Geometry: final body of the model. Coordinates: model frame, mm. Face numbers are marked on the shaded views. A direction names the side the tool comes from. Give positions to 0.01 mm unless a question says otherwise; leave off trailing zeros. Loops run counter-clockwise (first coordinate to the right, second up) from the corner with the lowest first, then second, coordinate; pieces in that order, holes last. Notation, with made-up numbers: (17.5, 0.5) -> (26.5, 0.5) arc R26 ccw to (26.5, 36.5) -> close; hole circle Ø2 at (34, 54). An arc over 180 degrees is marked (long way). One line per question, with ' | ' between items. Start each with the question number.
Item 1: Section D-D on z = 71.5. Return loops of the section in (x, y), then the cut area to 3 significant figures.
Item 2: Mould query, pull axis X, two halves, no side actions, for the marked faces 3, 4, 5 and 6. Classes: released by +X, released by -X, zero draft, split by the parting line, or undercut.
Item 3: Pin query (flat end, axial travel): P1, Ø3, axis at y = 7, z = 33, coming from the +X side; P2, Ø3, axis at x = -2.5, z = 8, coming from the +Y side; P3, Ø6, axis at x = -5.5, z = 41, coming from the -Y side; P4, Ø5, axis at x = 0, y = 0, coming from the +Z side. Return the tip coordinate at first contact, or that it passes through.
Item 4: Section C-C on z = 39.5. Return loops of the section in (x, y).
Item 5: Material intervals for line 1 along Y through (x, z) = (0, 45); line 2 along Z through (x, y) = (2.5, -7.25); line 3 along Y through (x, z) = (0, 70.75), sorted ascending. Write a range as [from, to].
Item 6: Section B-B on z = 6. Return loops of the section in (x, y).
Item 7: Set-up query: the marked faces 1 and 2. Return all of +Z, -Z, +X, -X, +Y, -Y with unobstructed straight access to the full face (end or side cutting, diameter ignored); none if empty.
from build123d import *

# Parameters (mm, degrees)
SKETCH_1_R                 = 10
EXTRUDE_1_DEPTH            = 70
SKETCH_2_R                 = 5
EXTRUDE_2_DEPTH            = 10.5
SKETCH_3_W                 = 0.75
SKETCH_3_H                 = 2.5
SKETCH_4_R                 = 1.5
CUT_EXTRUDE_1_DEPTH        = 15.5
HOLE_WIZARD_6_0_6_1_REACH  = 68.521
HOLE_WIZARD_6_0_6_1_BORE_R = 3
CHAMFER_1_SIZE             = 0.5
SKETCH_9_W                 = 10
SKETCH_9_H                 = 12
CUT_EXTRUDE_2_DEPTH        = 1.5


with BuildPart() as part:
    # 草图1 → 凸台-拉伸1 (new body)
    with BuildSketch(Plane.XY):
        Circle(SKETCH_1_R)
    extrude(amount=EXTRUDE_1_DEPTH)

    # 草图2 → 凸台-拉伸2 (add)
    with BuildSketch(Plane.XY.offset(70)):
        with Locations(Location((0, 0, 0), (0, 0, 180))):
            Circle(SKETCH_2_R)
    extrude(amount=EXTRUDE_2_DEPTH)

    # 草图3 → 切除-旋转1 (revolve, cut)
    with BuildSketch(Plane(origin=(0, 0, 0), x_dir=(1, 0, 0), z_dir=(0, 1, 0)), mode=Mode.PRIVATE) as cut_revolve_1_sk:
        with Locations((-4.625, -71.25)):
            Rectangle(SKETCH_3_W, SKETCH_3_H)
    revolve(cut_revolve_1_sk.sketch.rotate(Axis((0, 0, 80.5), (0, 0, -1)), 180), axis=Axis((0, 0, 80.5), (0, 0, -1)), mode=Mode.SUBTRACT)

    # 草图4 → 切除-拉伸1 (cut)
    with BuildSketch(Plane.XY.offset(80.5)):
        Circle(SKETCH_4_R)
    extrude(amount=-CUT_EXTRUDE_1_DEPTH, mode=Mode.SUBTRACT)

    # 草图5 → 1/4 NPT 螺纹孔1 (revolve, cut)
    with BuildSketch(Plane.YZ):
        Polygon((0, 0), (0, 20.412347279), (5.5626, 17.07), (5.5626, 10.02), (5.943676082, 10.02), (6.2436883, 0), align=None)
    revolve(axis=Axis((0, 0, -6.35), (0, 0, 1)), mode=Mode.SUBTRACT)

    # Ø6.0 (6) 直径孔1 bore → Ø6.0 (6) 直径孔1 (cut, up to next)
    with BuildSketch(Plane.XY.offset(65), mode=Mode.PRIVATE) as hole_wizard_6_0_6_1_sk1:
        Circle(HOLE_WIZARD_6_0_6_1_BORE_R)
    hole_wizard_6_0_6_1_tool1 = extrude(hole_wizard_6_0_6_1_sk1.sketch, amount=-HOLE_WIZARD_6_0_6_1_REACH, mode=Mode.PRIVATE) & part.part
    add(hole_wizard_6_0_6_1_tool1.solids().sort_by_distance((0, 0, 65))[0], mode=Mode.SUBTRACT)

    # 倒角1
    chamfer_1_edges = [part.edges().sort_by_distance(p)[0] for p in [
        (-10, 0, 0),
        (-10, 0, 70),
        (5, 0, 80.5),
    ]]
    chamfer(chamfer_1_edges, length=CHAMFER_1_SIZE)

    # 草图9 → 切除-拉伸2 (cut)
    with BuildSketch(Plane(origin=(0, 10, 0), x_dir=(1, 0, 0), z_dir=(0, 1, 0))):
        with Locations((0, -6)):
            Rectangle(SKETCH_9_W, SKETCH_9_H)
    cut_extrude_2 = extrude(amount=-CUT_EXTRUDE_2_DEPTH, mode=Mode.SUBTRACT)

    # 镜向1: 切除-拉伸2 across plane
    add(cut_extrude_2.mirror(Plane.ZX), mode=Mode.SUBTRACT)


solid = part.part
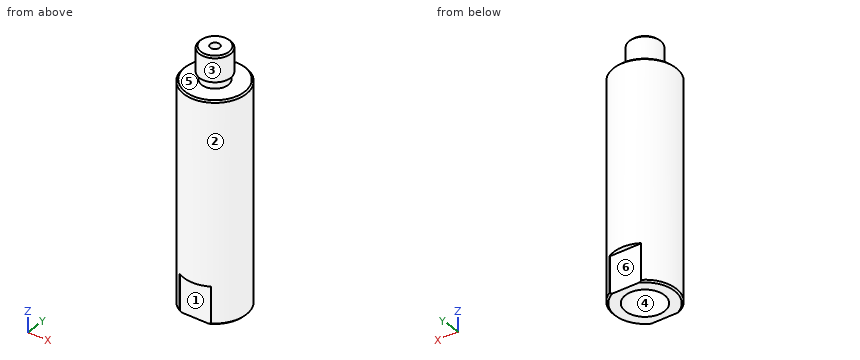
Result sheet:
1) outline: circle Ø8.5 at (0, 0); hole circle Ø3 at (0, 0) | area: 49.7 mm²
2) face 3: split by the parting line | face 4: undercut | face 5: zero draft | face 6: undercut
3) P1: stops at x = 8.35 | P2: stops at y = 8.5 | P3: stops at y = -9.68 | P4: stops at z = 80.5
4) outline: circle Ø20 at (0, 0); hole circle Ø6 at (0, 0)
5) line 1: y = [-10, -3], [3, 10] | line 2: z = [0, 70] | line 3: y = [-4.25, -1.5], [1.5, 4.25]
6) outline: (-5, -8.66) -> (-5, -8.5) -> (5, -8.5) -> (5, -8.66) arc R10 ccw to (5, 8.66) -> (5, 8.5) -> (-5, 8.5) -> (-5, 8.66) arc R10 ccw to start; hole circle Ø12.13 at (0, 0)
7) face 1: -Z, -Y | face 2: +Z, -Z
